from build123d import *

# Parameters (mm, degrees)
SKETCH_1_R                = 20
EXTRUDE_1_DEPTH           = 3
EXTRUDE_1_TAPER           = -20
EXTRUDE_1_OTHER_WAY_DEPTH = 2
SKETCH_2_R                = 18
CUT_EXTRUDE_START         = 34
SKETCH_5_R                = 37.541334734
CUT_EXTRUDE_1_DEPTH       = 53
SHELL_1_T                 = -1


with BuildPart() as part:
    # 草图1 → 凸台-拉伸1 (new body)
    with BuildSketch(Plane.XY):
        Circle(SKETCH_1_R)
    extrude(amount=EXTRUDE_1_DEPTH, taper=EXTRUDE_1_TAPER)

    # 草图1 → 凸台-拉伸1 other way (add)
    with BuildSketch(Plane.XY):
        Circle(SKETCH_1_R)
    extrude(amount=-EXTRUDE_1_OTHER_WAY_DEPTH)

    # 扫描1: sweep along a path in 草图3
    with BuildLine(Plane(origin=(0, 0, 0), x_dir=(0, 0, -1), z_dir=(1, 0, 0))) as sweep_1_path:
        Line((2, 0), (46.016642033, -9.356026087))
    # 草图2 → 扫描1 (sweep)
    with BuildSketch(Plane(origin=(0, 0, -2), x_dir=(-1, 0, 0), z_dir=(0, 0, -1))):
        Circle(SKETCH_2_R)
    sweep(path=sweep_1_path.line)

    # 草图5 → 切除-拉伸1 (cut)
    with BuildSketch(Plane(origin=(0, 0, -2), x_dir=(-1, 0, 0), z_dir=(0, 0, -1)).offset(CUT_EXTRUDE_START)):
        Circle(SKETCH_5_R)
    extrude(amount=CUT_EXTRUDE_1_DEPTH, mode=Mode.SUBTRACT)

    # 抽壳1
    shell_1_openings = [part.faces().sort_by_distance(p)[0] for p in [
        (0, 0, 3),
        (-1.512e-06, -7.226932051, -36),
    ]]
    offset(amount=SHELL_1_T, openings=shell_1_openings, kind=Kind.INTERSECTION)


solid = part.part
Model file for the job. Use its own axes, mm. A direction names the side the tool comes from. Give positions to 0.01 mm unless a question says otherwise; leave off trailing zeros. Answer as CSV lines item,"result".
1. Two-plate mould, pull along X, no slides. Class faces 1 (the face through (-4.336, -19.524, -0.986)), 2 (the face through (8.767, -16.856, -0.404)), 3 (the face through (-13, 4, -36)): +X half, -X half, draft (parallel to the pull), parting line (faces both ways), or undercut.
Responses:
face 1,"parting line"
face 2,"undercut"
face 3,"draft"
2. Pin check, flat tips, straight feed: pin 1 (1.5 mm diameter, centred on y = -15, z = -32, fed in from -X); pin 2 (5 mm diameter, centred on y = -19, z = -2, fed in from +X); pin 3 (3 mm diameter, centred on x = -4.5, z = -16, fed in from +Y). Stop position of each tip, or through.
Responses:
pin 1,"stops at x = -16.19"
pin 2,"stops at x = 11.3"
pin 3,"stops at y = 14.92"
3. 3-axis set-ups, long thin cutter, end or side, ignore diameter. For faces 4 (the face through (-11, -13, -1)), 5 (the face through (-18, 3, -2)), 6 (the face through (19, -8, 3)): which of +Z, -Z, +X, -X, +Y, -Y reach the whole face in a straight line?
Responses:
face 4,"+Z"
face 5,"none"
face 6,"+Z, +X, -X, +Y, -Y"
4. Drill centre lines: L1, parallel to Y at x = 0, z = 0; L2, parallel to Y at x = -3.5, z = -15.5; L3, parallel to X at y = 4, z = 0. Where is each one in solid material? Low to high. Write a range as [from, to].
Responses:
L1,"y = [-20, -19], [19, 20]"
L2,"y = [-20.53, -19.48], [13.74, 14.79]"
L3,"x = [-19.6, -18.57], [18.57, 19.6]"
